from build123d import *

# Parameters (mm, degrees)
BRACKET_BODY_DEPTH     = 60
CORNER_FILLET_R30_R    = 30
CORNER_FILLET_R20_R    = 20
BASE_NOTCH_DEPTH       = 78
UPRIGHT_SLOTS_3X_DEPTH = 20
BASE_BOSSES_PROFILE_R  = 8
BASE_BOSSES_2X_DEPTH   = 10
BOSS_EDGE_FILLET_R2_R  = 2
BOSS_HOLES_PROFILE_R   = 6
BOSS_HOLES_2X_DEPTH    = 10


with BuildPart() as part:
    # Bracket L Profile → Bracket Body (new, symmetric)
    with BuildSketch(Plane.XY):
        with BuildLine():
            Line((20, 0), (0, 0))
            Line((0, 0), (0, -80))
            Line((0, -80), (0, -100))
            Line((0, -100), (20, -100))
            Line((20, -100), (100, -100))
            Line((100, -100), (100, -80))
            Line((100, -80), (30, -80))
            ThreePointArc((30, -80), (22.928932188, -77.071067812), (20, -70))
            Line((20, -70), (20, 0))
        make_face()
    extrude(amount=BRACKET_BODY_DEPTH, both=True)

    # Corner Fillet R30
    corner_fillet_r30_edges = [part.edges().sort_by_distance(p)[0] for p in [
        (100, -90, 60),
        (100, -90, -60),
    ]]
    fillet(corner_fillet_r30_edges, radius=CORNER_FILLET_R30_R)

    # Corner Fillet R20
    corner_fillet_r20_edges = [part.edges().sort_by_distance(p)[0] for p in [
        (10, 0, -60),
        (10, 0, 60),
    ]]
    fillet(corner_fillet_r20_edges, radius=CORNER_FILLET_R20_R)

    # Base Notch Profile → Base Notch (cut)
    with BuildSketch(Plane(origin=(0, -80, 0), x_dir=(1, 0, 0), z_dir=(0, 1, 0))):
        with BuildLine():
            Line((65, 15), (100, 15))
            Line((100, 15), (100, -15))
            Line((100, -15), (65, -15))
            ThreePointArc((65, -15), (50, 0), (65, 15))
        make_face()
    extrude(amount=-BASE_NOTCH_DEPTH, mode=Mode.SUBTRACT)

    # Upright Slots Profile → Upright Slots 3x (cut)
    with BuildSketch(Plane(origin=(20, 0, 0), x_dir=(0, 0, -1), z_dir=(1, 0, 0))):
        with BuildLine():
            Line((-40, -14), (40, -14))
            ThreePointArc((40, -14), (46, -20), (40, -26))
            Line((40, -26), (-40, -26))
            ThreePointArc((-40, -26), (-46, -20), (-40, -14))
        make_face()
        with BuildLine():
            Line((-40, -46), (40, -46))
            ThreePointArc((40, -46), (46, -40), (40, -34))
            Line((40, -34), (-40, -34))
            ThreePointArc((-40, -34), (-46, -40), (-40, -46))
        make_face()
        with BuildLine():
            Line((-40, -66), (40, -66))
            ThreePointArc((40, -66), (46, -60), (40, -54))
            Line((40, -54), (-40, -54))
            ThreePointArc((-40, -54), (-46, -60), (-40, -66))
        make_face()
    extrude(amount=-UPRIGHT_SLOTS_3X_DEPTH, mode=Mode.SUBTRACT)

    # Base Bosses Profile → Base Bosses 2x (add)
    with BuildSketch(Plane(origin=(0, -80, 0), x_dir=(1, 0, 0), z_dir=(0, 1, 0))):
        with Locations(Location((70, 30, 0), (0, 0, 270))):
            Circle(BASE_BOSSES_PROFILE_R)
        with Locations(Location((70, -30, 0), (0, 0, 270))):
            Circle(BASE_BOSSES_PROFILE_R)
    extrude(amount=BASE_BOSSES_2X_DEPTH)

    # Boss Edge Fillet R2
    boss_edge_fillet_r2_edges = [part.edges().sort_by_distance(p)[0] for p in [
        (70, -80, -38),
        (70, -80, 22),
    ]]
    fillet(boss_edge_fillet_r2_edges, radius=BOSS_EDGE_FILLET_R2_R)

    # Boss Holes Profile → Boss Holes 2x (cut)
    with BuildSketch(Plane(origin=(0, -70, 0), x_dir=(1, 0, 0), z_dir=(0, 1, 0))):
        with Locations(Location((70, -30, 0), (0, 0, 270))):
            Circle(BOSS_HOLES_PROFILE_R)
        with Locations(Location((70, 30, 0), (0, 0, 270))):
            Circle(BOSS_HOLES_PROFILE_R)
    extrude(amount=-BOSS_HOLES_2X_DEPTH, mode=Mode.SUBTRACT)


solid = part.part
The model under review builds one solid part; all positions refer to its coordinate system, in mm. A direction names the side the tool comes from. Round coordinates to 2 decimals unless told otherwise and drop trailing zeros. Order: outer loops, then holes, each group sorted by start corner. A loop starts at its lowest first (then second) coordinate and runs counter-clockwise, first axis right, second up. Notation, with made-up numbers: (7.5, -23) -> (12.5, -23) arc R20 cw to (12.5, -8) -> close; hole circle Ø7 at (-4, 9). An arc over 180 degrees is marked (long way). Write item = value, one per line. Start each with the question number.
Item 1: For line 1 along Y through (x, z) = (11, -21); line 2 along X through (y, z) = (-75, 30); line 3 along Z through (x, y) = (71.5, -74), list the stretches that pass through material, from the lowest coordinate up.
Item 2: Consider section D-D on x = 87.5. Write out the cut boundary in (y, z).
Item 3: Clearance check with flat-ended pins moving along their axes: pin 1 Ø21 at (x, z) = (59.5, 26) entering from +Y; pin 2 Ø10 at (x, y) = (10.5, -14.5) entering from +Z; pin 3 Ø10 at (x, y) = (90.5, -85) entering from -Z; pin 4 Ø1 at (y, z) = (-56, 10) entering from +X. State where each tip first meets the part, or that it passes through.
Item 4: Consider section C-C on y = -60. Write out the cut boundary in (x, z).
Item 5: Mouldability with a two-part tool opening along Y and no side actions: class faces 1 (the face through (0, -49, 1)), 2 (the face through (10, -46, 1)), 3 (the face through (10, -26, -1)), 4 (the face through (9.86, -6.014, 54.297)) as released by +Y, released by -Y, zero draft, split by the parting line, or undercut.
Item 6: Consider section B-B on y = -75. Write out the cut boundary in (x, z), plus the area to 3 significant figures.
Item 7: Consider section A-A on z = -17.5. Write out the cut boundary in (x, y).
Item 8: For faces 5 (the face through (77.932, -74.056, 28.959)), 6 (the face through (23.01, -77.15, 0.84)), 7 (the face through (10, -40, 46)), 8 (the face through (82, -90, -15)), list the 3-axis set-ups (+Z, -Z, +X, -X, +Y, -Y) from which the entire face can be reached by the end or side of a thin tool; tool diameter is ignored.
Conclusion:
q1.line_1 = -100 to -66, -54 to -46, -34 to -26, -14 to 0
q1.line_2 = 0 to 21.34, 62 to 64, 76 to 78
q1.line_3 = -37.86 to -35.81, -24.19 to -22.14, 22.14 to 24.19, 35.81 to 37.86
q2.outline = (-100, -54.37) -> (-80, -54.37) -> (-80, -15) -> (-100, -15) -> close; (-100, 15) -> (-80, 15) -> (-80, 54.37) -> (-100, 54.37) -> close
q3.pin_1 = -70
q3.pin_2 = 59.99
q3.pin_3 = -55.69
q3.pin_4 = through
q4.outline = (0, -60) -> (20, -60) -> (20, -46) -> (0, -46) -> close; (0, 46) -> (20, 46) -> (20, 60) -> (0, 60) -> close
q5.face_1 = zero draft
q5.face_2 = undercut
q5.face_3 = undercut
q5.face_4 = released by +Y
q6.outline = (0, -60) -> (21.34, -60) -> (21.34, 60) -> (0, 60) -> close; circle Ø16 at (70, -30); circle Ø16 at (70, 30); hole circle Ø12 at (70, -30); hole circle Ø12 at (70, 30)
q6.area = 2,740 mm2
q7.outline = (0, -100) -> (100, -100) -> (100, -80) -> (30, -80) arc R10 cw to (20, -70) -> (20, -66) -> (0, -66) -> close; (0, -54) -> (20, -54) -> (20, -46) -> (0, -46) -> close; (0, -34) -> (20, -34) -> (20, -26) -> (0, -26) -> close; (0, -14) -> (20, -14) -> (20, 0) -> (0, 0) -> close
q8.face_5 = +Y
q8.face_6 = +Z, -Z, +Y
q8.face_7 = +X, -X
q8.face_8 = +X, +Y, -Y
